```python
from build123d import *

# Parameters (mm, degrees)
EXTRUDE_1_DEPTH              = 12.5
HOLE_WIZARD_M4_1_D           = 3.3
HOLE_WIZARD_M4_1_DEPTH       = 9.5
HOLE_WIZARD_M4_1_TIP         = 0.991420021
HOLE_WIZARD_M6_1_D           = 5
HOLE_WIZARD_M6_1_DEPTH       = 12
HOLE_WIZARD_M6_1_CSINK_D     = 6.05
HOLE_WIZARD_M6_1_CSINK_ANGLE = 90
HOLE_WIZARD_M6_1_TIP         = 1.502151548


with BuildPart() as part:
    # 草图1 → 凸台-拉伸1 (new, symmetric)
    with BuildSketch(Plane.XY):
        with BuildLine():
            Line((-27, 65.5), (27, 65.5))
            Line((27, 65.5), (27, -17))
            Line((27, -17), (9, -17))
            Line((9, -17), (9, -13.228756555))
            ThreePointArc((9, -13.228756555), (0, 16), (-9, -13.228756555))
            Line((-9, -13.228756555), (-9, -17))
            Line((-9, -17), (-27, -17))
            Line((-27, -17), (-27, 65.5))
        make_face()
    extrude(amount=EXTRUDE_1_DEPTH, both=True)

    # M4 螺纹孔1
    with Locations(Plane.XY.offset(12.5)):
        with Locations((18.186533479, 10.5), (18.186533479, -10.5), (-18.186533479, -10.5), (-18.186533479, 10.5)):
            Hole(HOLE_WIZARD_M4_1_D / 2, depth=HOLE_WIZARD_M4_1_DEPTH)
            with Locations((0, 0, -(HOLE_WIZARD_M4_1_DEPTH + HOLE_WIZARD_M4_1_TIP / 2))):  # 118° drill point
                Cone(0, HOLE_WIZARD_M4_1_D / 2, HOLE_WIZARD_M4_1_TIP, mode=Mode.SUBTRACT)

    # M6 螺纹孔1
    with Locations(Plane(origin=(-20, 65.5, 5.5), x_dir=(0, 0, 1), z_dir=(0, 1, 0))):
        with Locations((0, 0), (-11, 0), (-11, 40), (0, 40)):
            CounterSinkHole(HOLE_WIZARD_M6_1_D / 2, HOLE_WIZARD_M6_1_CSINK_D / 2, depth=HOLE_WIZARD_M6_1_DEPTH, counter_sink_angle=HOLE_WIZARD_M6_1_CSINK_ANGLE)
            with Locations((0, 0, -(HOLE_WIZARD_M6_1_DEPTH + HOLE_WIZARD_M6_1_TIP / 2))):  # 118° drill point
                Cone(0, HOLE_WIZARD_M6_1_D / 2, HOLE_WIZARD_M6_1_TIP, mode=Mode.SUBTRACT)


solid = part.part
```
Design review of the part built by this model. Coordinates are the model's own, in mm. A direction names the side the tool comes from. Give positions to 0.01 mm unless a question says otherwise; leave off trailing zeros. Order: outer loops, then holes, each group sorted by start corner. A loop starts at its lowest first (then second) coordinate and runs counter-clockwise, first axis right, second up. Notation, with made-up numbers: M -26,51 L 33,51 A14 cw 33,78 Z; hole C 60,-15.75 d3. An arc over 180 degrees is marked long. One line per question, with ' | ' between items. Start each with the question number.
Q1. The part is to be moulded in two halves that separate along X. For faces 4 (the face through (27, 25, 0)), 5 (the face through (-18, -17, 0)), 6 (the face through (18.15, -10.22, 2.18)), say which applies: +X half, -X half, draft (parallel to the pull), parting line (faces both ways), or undercut.
Q2. We need section D-D (x = -13). Write out the cut boundary in (y, z).
Q3. For L1, parallel to X at y = 61.25, z = 5.5; L2, parallel to Z at x = -20, y = 56.5; L3, parallel to Y at x = 18, z = 9, list the stretches that pass through material, from the lowest coordinate up. Write a range as [from, to].
Q4. Machinability: for faces 1 (the face through (-19.71, -11.13, 7.68)), 2 (the face through (22, 59, -7)), 3 (the face through (0, 34, -12.5)), which of the approach directions +Z, -Z, +X, -X, +Y, -Y give a long, thin tool a straight path to every point of the face, cutting with its end or side? Answer none if there is none.
Q5. We need section B-B (x = 11). Write out the cut boundary in (y, z).
Q6. For pin 1 Ø8 at (x, z) = (20, 5.5) entering from +Y; pin 2 Ø4.5 at (x, z) = (-20, 5.5) entering from +Y; pin 3 Ø5 at (x, z) = (-2.5, 8.5) entering from -Y, all flat-tipped, find the tip position at first contact; note any pin that passes through.
Q7. We need section A-A (y = 56.5). Write out the cut boundary in (x, z).
Q8. We need section C-C (z = 10). Write out the cut boundary in (x, y).
Returned:
1) face 4: +X half | face 5: draft | face 6: undercut
2) outline: M -17,-12.5 L -9.33,-12.5 L -9.33,12.5 L -17,12.5 Z; M 9.33,-12.5 L 65.5,-12.5 L 65.5,12.5 L 9.33,12.5 Z
3) L1: [-27, -22.5], [-17.5, 17.5], [22.5, 27] | L2: [-12.5, -8], [-3, 3], [8, 12.5] | L3: [-17, -12.14], [-8.86, 8.86], [12.14, 65.5]
4) face 1: +Z | face 2: +Y | face 3: -Z, +X, -X, +Y, -Y
5) outline: M -17,-12.5 L -11.62,-12.5 L -11.62,12.5 L -17,12.5 Z; M 11.62,-12.5 L 65.5,-12.5 L 65.5,12.5 L 11.62,12.5 Z
6) pin 1: y = 65.5 | pin 2: y = 53.35 | pin 3: y = 15.2
7) outline: M -27,-12.5 L 27,-12.5 L 27,12.5 L -27,12.5 Z; hole C -20,-5.5 d5; hole C -20,5.5 d5; hole C 20,-5.5 d5; hole C 20,5.5 d5
8) outline: M -27,-17 L -9,-17 L -9,-13.23 A16 cw long 9,-13.23 L 9,-17 L 27,-17 L 27,65.5 L -27,65.5 Z; hole C -18.19,-10.5 d3.3; hole C -18.19,10.5 d3.3; hole C 18.19,-10.5 d3.3; hole C 18.19,10.5 d3.3
